from build123d import *

# Parameters (mm, degrees)
SKETCH_1_W                   = 160
SKETCH_1_H                   = 150
EXTRUDE_1_DEPTH              = 10
FILLET_1_R                   = 5
HOLE_WIZARD_M6_1_D           = 6.6
HOLE_WIZARD_M6_1_DEPTH       = 11.5
HOLE_WIZARD_M6_1_CBORE_D     = 11
HOLE_WIZARD_M6_1_CBORE_DEPTH = 6.4
HOLE_WIZARD_M6_1_TIP         = 1.982840043
CUT_EXTRUDE_1_DEPTH          = 10


with BuildPart() as part:
    # 草图1 → 凸台-拉伸1 (new body)
    with BuildSketch(Plane.XY):
        with Locations((28963.620313483, 18.565660066)):
            Rectangle(SKETCH_1_W, SKETCH_1_H)
    extrude(amount=EXTRUDE_1_DEPTH)

    # 圆角1
    fillet_1_edges = [part.edges().sort_by_distance(p)[0] for p in [
        (28883.620313483, 93.565660066, 5),
        (29043.620313483, 93.565660066, 5),
        (29043.620313483, -56.434339934, 5),
        (28883.620313483, -56.434339934, 5),
    ]]
    fillet(fillet_1_edges, radius=FILLET_1_R)

    # M6 六角凹头螺钉的柱形沉头孔1
    with Locations(Plane(origin=(0, 0, 0), x_dir=(-1, 0, 0), z_dir=(0, 0, -1))):
        with Locations((-29024.620313483, 84.565660077), (-29024.620313483, 58.565660077), (-29024.620313483, -11.434339923), (-29024.620313483, -37.434339923), (-28902.620313482, -37.434339923), (-28902.620313482, -11.434339923), (-28902.620313482, 58.565660077), (-28902.620313482, 84.565660077)):
            CounterBoreHole(HOLE_WIZARD_M6_1_D / 2, HOLE_WIZARD_M6_1_CBORE_D / 2, HOLE_WIZARD_M6_1_CBORE_DEPTH, depth=HOLE_WIZARD_M6_1_DEPTH)
            with Locations((0, 0, -(HOLE_WIZARD_M6_1_DEPTH + HOLE_WIZARD_M6_1_TIP / 2))):  # 118° drill point
                Cone(0, HOLE_WIZARD_M6_1_D / 2, HOLE_WIZARD_M6_1_TIP, mode=Mode.SUBTRACT)

    # 草图4 → 切除-拉伸1 (cut)
    with BuildSketch(Plane.XY.offset(10)):
        with BuildLine():
            Line((28923.620313483, -1.434339933), (28923.620313483, 38.565660067))
            ThreePointArc((28923.620313483, 38.565660067), (28963.620313483, 78.565660067), (29003.620313483, 38.565660067))
            Line((29003.620313483, 38.565660067), (29003.620313483, -1.434339933))
            ThreePointArc((29003.620313483, -1.434339933), (28963.620313483, -41.434339933), (28923.620313483, -1.434339933))
        make_face()
    extrude(amount=-CUT_EXTRUDE_1_DEPTH, mode=Mode.SUBTRACT)


solid = part.part
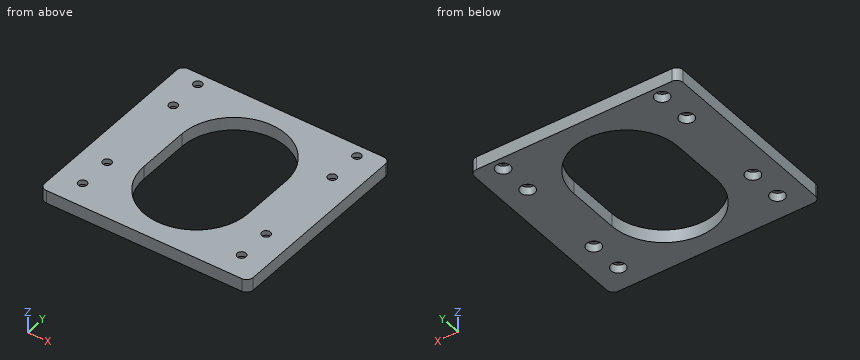
Design review of the part built by this model. Coordinates are the model's own, in mm. Coordinates: 2 decimals unless noted, no trailing zeros. Loops run counter-clockwise (first coordinate to the right, second up) from the corner with the lowest first, then second, coordinate; pieces in that order, holes last. Notation, with made-up numbers: M 3,-16 L 28,-16 A24 cw 28,20 Z; hole C 26.25,-32 d4. An arc over 180 degrees is marked long. Use one line per item in the form item = value.
(1) For line 1 along Y through (x, z) = (29024.5, 5.5); line 2 along X through (y, z) = (23, 2); line 3 along X through (y, z) = (-13, 2), list the stretches that pass through material, from the lowest coordinate up. Write a range as from..to.
Return value:
line_1 = -56.43..-42.93, -31.94..-16.93, -5.94..53.07, 64.06..79.07, 90.06..93.57
line_2 = 28883.62..28923.62, 29003.62..29043.62
line_3 = 28883.62..28897.35, 28907.89..28925.33, 29001.91..29019.35, 29029.89..29043.62
(2) Consider section A-A (y = 16). Write out the cut boundary in (x, z), and give its area (3 significant figures).
Return value:
outline = M 28883.62,0 L 28923.62,0 L 28923.62,10 L 28883.62,10 Z; M 29003.62,0 L 29043.62,0 L 29043.62,10 L 29003.62,10 Z
area = 800 mm2
(3) Consider section C-C (z = 8). Give the number of separate pieces and of enclosed holes in the cut face, and give its area (3 significant figures).
Return value:
separate_pieces = 1
enclosed_holes = 9
area = 15,500 mm2
(4) Clearance check with flat-ended pins moving along their axes: P1, Ø5.5, axis at x = 29024.62, y = -11.43, coming from the +Z side; P2, Ø5.5, axis at x = 28901.5, y = 84.5, coming from the -Z side. State where each tip first meets the part, or that it passes through.
Return value:
P1 = through
P2 = 6.4
(5) Consider section B-B (x = 28967). Write out the cut boundary in (y, z).
Return value:
outline = M -56.43,0 L -41.29,0 L -41.29,10 L -56.43,10 Z; M 78.42,0 L 93.57,0 L 93.57,10 L 78.42,10 Z
